```python
from build123d import *


with BuildPart() as part:
    # Bush Profile Sketch → Bush Body (revolve)
    with BuildSketch(Plane.XY, mode=Mode.PRIVATE) as bush_body_sk:
        Polygon((0, 10), (-4, 6), (-38, 6), (-42, 10), (-42, 16), (0, 16), align=None)
    revolve(bush_body_sk.sketch.rotate(Axis((0, 0, 0), (-1, 0, 0)), 90), axis=Axis((0, 0, 0), (-1, 0, 0)))

    # Internal Cut Profile Sketch → Internal Revolved Cut (revolve, cut)
    with BuildSketch(Plane.XY, mode=Mode.PRIVATE) as internal_revolved_cut_sk:
        Polygon((-26.196152423, -16), (-21, -13), (-21, -16), align=None)
    revolve(internal_revolved_cut_sk.sketch.rotate(Axis((-21, 0, 0), (0, -1, 0)), 180), axis=Axis((-21, 0, 0), (0, -1, 0)), mode=Mode.SUBTRACT)


solid = part.part
```
Geometry check sheet. Reference: the model listing, model coordinates, mm. Round coordinates to 2 decimals unless told otherwise and drop trailing zeros. Loops run counter-clockwise (first coordinate to the right, second up) from the corner with the lowest first, then second, coordinate; pieces in that order, holes last. Notation, with made-up numbers: (66, -21.5) - (119, -21.5) arc R20 ccw to (119, 17.5) - close; hole circle Ø3 at (54, 35). An arc over 180 degrees is marked (long way). Use a Markdown table: item, result.
Q1. Draft check along Z on faces 1 (the cylindrical face through (-20.71, 15.62, 3.47)), 2 (the flat face through (-42, -0.2, 10.4)), 3 (the conical face through (-38.25, 6.1, 1.35)). Enter one of: released by +Z, released by -Z, zero draft, split by the parting line, or undercut.
Solutions:
| item | result |
|---|---|
| face 1 | split by the parting line |
| face 2 | zero draft |
| face 3 | undercut |
Q2. Material ranges on line 1 (Y direction, x = -27, z = 0); line 2 (Y direction, x = -23, z = 0); line 3 (Z direction, x = -36, y = -2.5), recorded low to high.
Solutions:
| item | result |
|---|---|
| line 1 | y = -16 to -6, 6 to 16 |
| line 2 | y = -14.15 to -6, 6 to 16 |
| line 3 | z = -15.8 to -5.45, 5.45 to 15.8 |
Q3. Cross-section at A-A on y = 0. Record the cut outline in (x, z).
Solutions:
| item | result |
|---|---|
| outline | (-42, -16) - (0, -16) - (0, -10) - (-4, -6) - (-38, -6) - (-42, -10) - close; (-42, 10) - (-38, 6) - (-4, 6) - (0, 10) - (0, 16) - (-42, 16) - close |
Q4. Cross-section at D-D on y = 13.5. Record the cut outline in (x, z), plus the area to 3 significant figures.
Solutions:
| item | result |
|---|---|
| outline | (-42, -8.59) - (0, -8.59) - (0, 8.59) - (-42, 8.59) - close |
| area | 721 mm2 |
Q5. Go/stop test with flat-tipped pins: P1, Ø1, axis at y = -2.5, z = 9, coming from the -X side; P2, Ø3, axis at y = 2.5, z = -4, coming from the +X side; P3, Ø8, axis at x = -36, z = 5.5, coming from the -Y side. Record where each tip stops, or that it passes through.
Solutions:
| item | result |
|---|---|
| P1 | stops at x = -41.84 |
| P2 | stops at x = -3.78 |
| P3 | stops at y = -15.93 |
Q6. Cross-section at B-B on x = -11.5. Record the cut outline in (y, z).
Solutions:
| item | result |
|---|---|
| outline | circle Ø32 at (0, 0); hole circle Ø12 at (0, 0) |
Q7. Cross-section at C-C on z = -12. Record the cut outline in (x, y), plus the area to 3 significant figures.
Solutions:
| item | result |
|---|---|
| outline | (-42, -10.58) - (0, -10.58) - (0, 10.58) - (-42, 10.58) - close |
| area | 889 mm2 |
